Build history of the part. All positions in model axes, mm. A direction names the side the tool comes from. Round coordinates to 2 decimals unless told otherwise and drop trailing zeros. Write each loop counter-clockwise with the first axis right and the second up, starting at its lowest first coordinate (ties: lowest second). Pieces come first, ordered by that corner, then holes. Notation, with made-up numbers: (53.5, 67.5) -> (95.5, 67.5) arc R12 cw to (95.5, 72.5) -> close; hole circle Ø3 at (19, -32). An arc over 180 degrees is marked (long way). One line per question, with ' | ' between items.
from build123d import *

# Parameters (mm, degrees)
BASE_CYLINDER_SKETCH_19_05_R = 9.525
BASE_CYLINDER_19_05_DEPTH    = 14.06
TAPER_TOP_SKETCH_12_7_R      = 6.35
SHANK_SKETCH_R               = 6.35
SHANK_12_7_DEPTH             = 16.94
SHANK_FLAT_SKETCH_W          = 1.59
SHANK_FLAT_SKETCH_H          = 11.43
SHANK_FLAT_DEPTH             = 8.47
BORE_SKETCH_11_11_R          = 6.35
BORE_11_11_DEPTH             = 14.06
CROSS_HOLE_SKETCH_2_38_R     = 1.19
CROSS_HOLE_2_38_DEPTH        = 14.06


with BuildPart() as part:
    # Base Cylinder Sketch Ø19.05 → Base Cylinder Ø19.05 (new body)
    with BuildSketch(Plane(origin=(0, 0, 0), x_dir=(1, 0, 0), z_dir=(0, 1, 0))):
        with Locations(Location((0, 0, 0), (0, 0, 270))):
            Circle(BASE_CYLINDER_SKETCH_19_05_R)
    extrude(amount=BASE_CYLINDER_19_05_DEPTH)

    # Taper Top Sketch Ø12.7 → section 0 of taper_loft
    with BuildSketch(Plane(origin=(0, 21.16, 0), x_dir=(1, 0, 0), z_dir=(0, 1, 0)), mode=Mode.PRIVATE) as taper_loft_s0:
        Circle(TAPER_TOP_SKETCH_12_7_R)
    # loft up to a face of the part (taper_loft)
    loft([taper_loft_s0.sketch, Face(Wire([part.edges().sort_by_distance((6.943426176, 14.06, -6.520311184))[0]]))])

    # Shank Sketch → Shank Ø12.7 (add)
    with BuildSketch(Plane(origin=(0, 21.16, 0), x_dir=(1, 0, 0), z_dir=(0, 1, 0))):
        with Locations(Location((0, 0, 0), (0, 0, 270))):
            Circle(SHANK_SKETCH_R)
    extrude(amount=SHANK_12_7_DEPTH)

    # Shank Flat Sketch → Shank Flat (cut, symmetric)
    with BuildSketch(Plane.XY):
        with Locations((5.555, 32.385)):
            Rectangle(SHANK_FLAT_SKETCH_W, SHANK_FLAT_SKETCH_H)
    extrude(amount=SHANK_FLAT_DEPTH, both=True, mode=Mode.SUBTRACT)

    # Bore Sketch Ø11.11 → Bore Ø11.11 (cut)
    with BuildSketch(Plane.XZ):
        with Locations(Location((0, 0, 0), (0, 0, 270))):
            Circle(BORE_SKETCH_11_11_R)
    extrude(amount=-BORE_11_11_DEPTH, mode=Mode.SUBTRACT)

    # Cross Hole Sketch Ø2.38 → Cross Hole Ø2.38 (cut)
    with BuildSketch(Plane(origin=(0, 0, 0), x_dir=(0, 0, -1), z_dir=(1, 0, 0))):
        with Locations(Location((0, 6.38, 0), (0, 0, 180))):
            Circle(CROSS_HOLE_SKETCH_2_38_R)
    extrude(amount=CROSS_HOLE_2_38_DEPTH, mode=Mode.SUBTRACT)


solid = part.part
(1) Wall check: line 1 (Z direction, x = 7.4, y = 6.38); line 2 (X direction, y = 10, z = -4.5); line 3 (Y direction, x = -4.25, z = 4.5). Give the ranges that are in metal, low to high. Write a range as from..to.
Calculated:
line 1: -6..-1.19, 1.19..6 | line 2: -8.39..-4.48, 4.48..8.39 | line 3: 14.06..38.1
(2) Slice it at A-A (x = 0). Write the cut outline in (y, z) (3 decimals), then the cut area to 3 significant figures.
Calculated:
outline: (0, -9.525) -> (14.06, -9.525) -> (21.16, -6.35) -> (38.1, -6.35) -> (38.1, 6.35) -> (21.16, 6.35) -> (14.06, 9.525) -> (0, 9.525) -> (0, 6.35) -> (14.06, 6.35) -> (14.06, -6.35) -> (0, -6.35) -> close | area: 417 mm2
(3) Slice it at B-B (y = 22). Write the cut outline in (x, z).
Calculated:
outline: circle Ø12.7 at (0, 0)
(4) Drop flat-ended pins along their axis: pin 1 (0.5 mm diameter, centred on x = 5.5, z = 0.5, fed in from +Y); pin 2 (2 mm diameter, centred on x = -3, y = 24, fed in from -Z); pin 3 (6 mm diameter, centred on y = 19, z = 6, fed in from -X). Give the stop position or say it passes through.
Calculated:
pin 1: y = 26.67 | pin 2: z = -6.03 | pin 3: x = -7.3
(5) Mould opens along Z. For faces 6 (the flat face through (0, 14.06, 0)), 7 (the conical face through (-1.42, 20.72, 6.39)), 8 (the flat face through (4.76, 32, 0)) say: pulls with the +Z half, pulls with the -Z half, needs draft (parallel to the pull), parting line crosses it, or undercut.
Calculated:
face 6: undercut | face 7: parting line crosses it | face 8: needs draft
(6) 3-axis set-ups, long thin cutter, end or side, ignore diameter. For faces 1 (the cylindrical face through (7.857, 7.436, 0.549)), 2 (the flat face through (-6.2, 0, 2)), 3 (the flat face through (5, 26.67, 0)), 4 (the cylindrical face through (-6.2, 6.93, 1.38)), 5 (the cylindrical face through (-6.2, 29.51, -1.38)): which of +Z, -Z, +X, -X, +Y, -Y reach the whole face in a straight line?
Calculated:
face 1: +X | face 2: +Z, -Z, +X, -X, -Y | face 3: +Z, -Z, +X, +Y | face 4: -Y | face 5: +Y
